The model under review builds one solid part; all positions refer to its coordinate system, in mm. A direction names the side the tool comes from. Give positions to 0.01 mm unless a question says otherwise; leave off trailing zeros. Order: outer loops, then holes, each group sorted by start corner. A loop starts at its lowest first (then second) coordinate and runs counter-clockwise, first axis right, second up.
```python
from build123d import *

# Parameters (mm, degrees)
SKETCH1_R                                            = 25
SKETCH1_R_2                                          = 18
BOSS_EXTRUDE1_DEPTH                                  = 35
SKETCH2_R                                            = 37.5
SKETCH2_R_2                                          = 18
BOSS_EXTRUDE2_DEPTH                                  = 10
HOLE_SIZE_PER_SOCKET_HEAD_CAP_SCREW_TYPE_D           = 4.5
HOLE_SIZE_PER_SOCKET_HEAD_CAP_SCREW_TYPE_CBORE_D     = 8
HOLE_SIZE_PER_SOCKET_HEAD_CAP_SCREW_TYPE_CBORE_DEPTH = 4.6


with BuildPart() as part:
    # Sketch1 → Boss-Extrude1 (new body)
    with BuildSketch(Plane.XY):
        Circle(SKETCH1_R)
        Circle(SKETCH1_R_2, mode=Mode.SUBTRACT)
    extrude(amount=BOSS_EXTRUDE1_DEPTH)

    # Sketch2 → Boss-Extrude2 (add)
    with BuildSketch(Plane.XY.offset(35)):
        Circle(SKETCH2_R)
        Circle(SKETCH2_R_2, mode=Mode.SUBTRACT)
    extrude(amount=BOSS_EXTRUDE2_DEPTH)

    # Hole size per socket head cap screw type3 (through all)
    with Locations(Plane.XY.offset(45)):
        with Locations((-8.588225841, -29.786614056), (8.588225841, 29.786614056)):
            CounterBoreHole(HOLE_SIZE_PER_SOCKET_HEAD_CAP_SCREW_TYPE_D / 2, HOLE_SIZE_PER_SOCKET_HEAD_CAP_SCREW_TYPE_CBORE_D / 2, HOLE_SIZE_PER_SOCKET_HEAD_CAP_SCREW_TYPE_CBORE_DEPTH)


solid = part.part
```
Item 1: For faces 1 (the cylindrical face through (23.846, 7.509, 17.255)), 2 (the flat face through (10.3, 28.1, 40.4)), 3 (the cylindrical face through (6.51, 28.92, 37.66)), list the 3-axis set-ups (+Z, -Z, +X, -X, +Y, -Y) from which the entire face can be reached by the end or side of a thin tool; tool diameter is ignored.
Values found:
face 1: -Z
face 2: +Z
face 3: +Z, -Z
Item 2: Clearance check with flat-ended pins moving along their axes: pin 1 Ø10 at (x, z) = (0, 12) entering from -Y; pin 2 Ø4 at (y, z) = (-5, 13.5) entering from +X; pin 3 Ø4 at (x, y) = (6.5, 29.5) entering from -Z. State where each tip first meets the part, or that it passes through.
Values found:
pin 1: stops at y = -25
pin 2: stops at x = 24.82
pin 3: stops at z = 35
Item 3: Take a section at D-D (x = 32). Give the boundary of the cut face in (y, z).
Values found:
outline: (-19.55, 35) - (19.55, 35) - (19.55, 45) - (-19.55, 45) - close
Item 4: Take a section at C-C (z = 16). Give the boundary of the cut face in (x, y).
Values found:
outline: circle Ø50 at (0, 0); hole circle Ø36 at (0, 0)
Item 5: Take a section at A-A (y = 0). Give the boundary of the cut face in (x, z), and give its area (3 significant figures).
Values found:
outline: (-37.5, 35) - (-25, 35) - (-25, 0) - (-18, 0) - (-18, 45) - (-37.5, 45) - close; (18, 0) - (25, 0) - (25, 35) - (37.5, 35) - (37.5, 45) - (18, 45) - close
area: 880 mm2
Item 6: For line 1 (Y direction, x = 0, z = 24); line 2 (Z direction, x = 23.5, y = -21); line 3 (Y direction, x = 1.5, z = 33), list the stretches that pass through material, from the lowest coordinate up.
Values found:
line 1: y = -25 to -18, 18 to 25
line 2: z = 35 to 45
line 3: y = -24.95 to -17.94, 17.94 to 24.95
Item 7: Draft analysis for pull direction Y (two halves, no side actions). For faces 4 (the flat face through (-7, -32, 40.4)), 5 (the cylindrical face through (-4.88, 37.18, 39.93)), 6 (the flat face through (16, 9, 45)), state which applies: released by +Y, released by -Y, zero draft, split by the parting line, or undercut.
Values found:
face 4: undercut
face 5: split by the parting line
face 6: zero draft
